from build123d import *

# Parameters (mm, degrees)
BOSS_EXTRUDE1_DEPTH = 5
SKETCH2_R           = 1.5
CUT_EXTRUDE1_DEPTH  = 15.5
CUT_EXTRUDE3_DEPTH  = 27
CIRPATTERN1_COUNT   = 3
CIRPATTERN2_COUNT   = 3
SCALE_RATIO_1_SCALE = 1.3
SKETCH5_R           = 5
CUT_EXTRUDE4_DEPTH  = 10
CHAMFER1_SIZE       = 0.5
SKETCH8_R           = 2
CUT_EXTRUDE5_DEPTH  = 10
CHAMFER2_SIZE       = 0.5
FILLET1_R           = 0.5


with BuildPart() as part:
    # Sketch1 → Boss-Extrude1 (new body)
    with BuildSketch(Plane.XY):
        with BuildLine():
            Line((-26.5, -17.60918321), (-12.640472866, -9.607381488))
            ThreePointArc((-12.640472866, -9.607381488), (-13.75, -7.938566201), (-14.640472866, -6.143279873))
            Line((-14.640472866, -6.143279873), (-28.5, -14.145081595))
            Line((-28.5, -14.145081595), (-29.75, -11.980018086))
            Line((-29.75, -11.980018086), (-15.436166994, -3.715922747))
            ThreePointArc((-15.436166994, -3.715922747), (-13.75, 7.938566201), (-4.5, 15.226074127))
            Line((-4.5, 15.226074127), (-4.5, 31.754264805))
            Line((-4.5, 31.754264805), (-2, 31.754264805))
            Line((-2, 31.754264805), (-2, 15.750661362))
            ThreePointArc((-2, 15.750661362), (0, 15.877132403), (2, 15.750661362))
            Line((2, 15.750661362), (2, 31.754264805))
            Line((2, 31.754264805), (4.5, 31.754264805))
            Line((4.5, 31.754264805), (4.5, 15.226074127))
            ThreePointArc((4.5, 15.226074127), (13.75, 7.938566201), (15.436166994, -3.715922747))
            Line((15.436166994, -3.715922747), (29.75, -11.980018086))
            Line((29.75, -11.980018086), (28.5, -14.145081595))
            Line((28.5, -14.145081595), (14.640472866, -6.143279873))
            ThreePointArc((14.640472866, -6.143279873), (13.75, -7.938566201), (12.640472866, -9.607381488))
            Line((12.640472866, -9.607381488), (26.5, -17.60918321))
            Line((26.5, -17.60918321), (25.25, -19.77424672))
            Line((25.25, -19.77424672), (10.936166994, -11.510151381))
            ThreePointArc((10.936166994, -11.510151381), (0, -15.877132403), (-10.936166994, -11.510151381))
            Line((-10.936166994, -11.510151381), (-25.25, -19.77424672))
            Line((-25.25, -19.77424672), (-26.5, -17.60918321))
        make_face()
    extrude(amount=BOSS_EXTRUDE1_DEPTH)

    # Sketch2 → Cut-Extrude1 (cut, symmetric)
    with BuildSketch(Plane(origin=(0, 0, 0), x_dir=(0, 0, -1), z_dir=(1, 0, 0))):
        with Locations(Location((-2.5, 21, 0), (0, 0, 90))):
            Circle(SKETCH2_R)
    cut_extrude1 = extrude(amount=CUT_EXTRUDE1_DEPTH, both=True, mode=Mode.SUBTRACT)

    # Sketch4 → Cut-Extrude3 (cut)
    with BuildSketch(Plane.ZY.offset(4.5)):
        with BuildLine():
            Line((0, 21), (0, 31.754264805))
            Line((0, 31.754264805), (5, 31.754264805))
            Line((5, 31.754264805), (5, 21))
            ThreePointArc((5, 21), (2.5, 23.5), (0, 21))
        make_face()
    cut_extrude3 = extrude(amount=-CUT_EXTRUDE3_DEPTH, mode=Mode.SUBTRACT)

    # CirPattern1: Cut-Extrude3 ×3 about axis
    cirpattern1_axis = Axis((0, 0, 5), (0, 0, -1))
    for i in range(1, CIRPATTERN1_COUNT):
        add(cut_extrude3.rotate(cirpattern1_axis, i * 360 / CIRPATTERN1_COUNT), mode=Mode.SUBTRACT)

    # CirPattern2: Cut-Extrude1 ×3 about axis
    cirpattern2_axis = Axis((0, 0, 5), (0, 0, -1))
    for i in range(1, CIRPATTERN2_COUNT):
        add(cut_extrude1.rotate(cirpattern2_axis, i * 360 / CIRPATTERN2_COUNT), mode=Mode.SUBTRACT)


with BuildPart() as part_1:
    # Scale ratio 1: scaled about (0, 0, 2.5)
    add(part.part.scale(SCALE_RATIO_1_SCALE).moved(Location((0, 0, -0.75))))

    # Sketch5 → Cut-Extrude4 (cut)
    with BuildSketch(Plane.XY.offset(5.75)):
        Circle(SKETCH5_R)
    extrude(amount=-CUT_EXTRUDE4_DEPTH, mode=Mode.SUBTRACT)

    # Chamfer1
    chamfer1_edges = [part_1.edges().sort_by_distance(p)[0] for p in [
        (-5, 0, -0.75),
        (-5, 0, 5.75),
    ]]
    chamfer(chamfer1_edges, length=CHAMFER1_SIZE)

    # Sketch8 → Cut-Extrude5 (cut)
    with BuildSketch(Plane.XY.offset(5.75)):
        with Locations((0, 15)):
            Circle(SKETCH8_R)
        with Locations((12.990381057, -7.5)):
            Circle(SKETCH8_R)
        with Locations((-12.990381057, -7.5)):
            Circle(SKETCH8_R)
    extrude(amount=-CUT_EXTRUDE5_DEPTH, mode=Mode.SUBTRACT)

    # Chamfer2
    chamfer2_edges = [part_1.edges().sort_by_distance(p)[0] for p in [
        (-2, 15, -0.75),
        (-2, 15, 5.75),
        (10.990381057, -7.5, -0.75),
        (10.990381057, -7.5, 5.75),
        (-14.990381057, -7.5, -0.75),
        (-14.990381057, -7.5, 5.75),
    ]]
    chamfer(chamfer2_edges, length=CHAMFER2_SIZE)

    # Fillet1
    fillet1_edges = [part_1.edges().sort_by_distance(p)[0] for p in [
        (-16.432614725, -12.489595935, 2.5),
        (-19.032614725, -7.986263835, 2.5),
        (-20.067017093, -4.830699571, 2.5),
        (-5.85, 19.793896366, 2.5),
        (-2.6, 20.47585977, 2.5),
        (2.6, 20.47585977, 2.5),
        (5.85, 19.793896366, 2.5),
        (20.067017093, -4.830699571, 2.5),
        (19.032614725, -7.986263835, 2.5),
        (16.432614725, -12.489595935, 2.5),
        (14.217017093, -14.963196795, 2.5),
        (-14.217017093, -14.963196795, 2.5),
    ]]
    fillet(fillet1_edges, radius=FILLET1_R)


solid = part_1.part
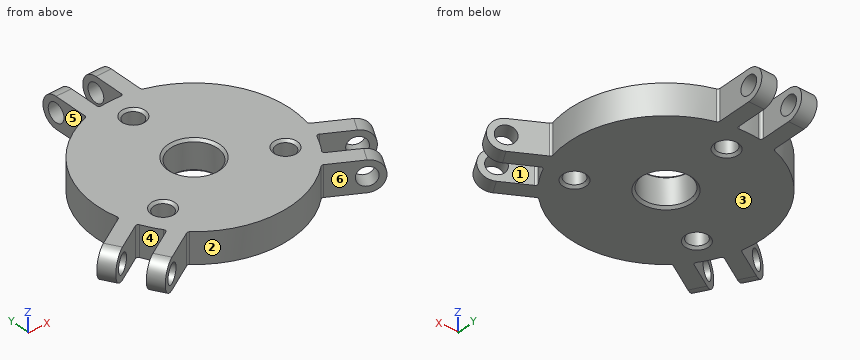
The listing builds one solid part. Answer for the finished solid, in the listing's coordinates (mm). Face numbers are marked on the shaded views. A direction names the side the tool comes from. Round coordinates to 2 decimals unless told otherwise and drop trailing zeros. Write each loop counter-clockwise with the first axis right and the second up, starting at its lowest first coordinate (ties: lowest second). Pieces come first, ordered by that corner, then holes. Notation, with made-up numbers: M -31,-7.5 L 7,-7.5 A21 ccw 7,29.5 Z; hole C 22,37 d2. An arc over 180 degrees is marked long. Write each question's results on one line, items separated by ' | '. Start each with the question number.
Item 1: A cutting plane is placed at A-A on x = 0. Write down the section's boundary in (y, z).
Item 2: A cutting plane is placed at C-C on y = 15. Write down the section's boundary in (x, z).
Item 3: A cutting plane is placed at B-B on y = 22.5. Write down the section's boundary in (x, z).
Item 4: For the marked faces 4, 5 and 6, determine the directions among +Z, -Z, +X, -X, +Y, -Y from which every point of the face is accessible in a straight line to the end or side of a thin tool.
Item 5: For a pull along Y with two mould halves and no side action, classify the marked faces 1, 2 and 3 as pulls with the +Y half, pulls with the -Y half, needs draft (parallel to the pull), parting line crosses it, or undercut.
Item 6: A cutting plane is placed at D-D on z = 3.5. State how many separate pieces and enclosed holes the cut face has, and give its area (3 significant figures).
Item 7: Straight lines are drawn through the part: L1, parallel to Y at x = 0, z = 2.8; L2, parallel to Y at x = 3, z = 3.5; L3, parallel to X at y = -11, z = 3.25. For each, find the intervals that lie inside material, in ascending order. Write a range as [from, to].
Item 8: Flat-ended cylindrical pins translate along their axes: pin 1 Ø3 at (y, z) = (27, 4) entering from -X; pin 2 Ø2.5 at (x, y) = (-12.99, -7.5) entering from -Z; pin 3 Ø2 at (y, z) = (-14, 5) entering from -X; pin 4 Ø11.5 at (x, y) = (0, 0) entering from -Z. Find the tip coordinate at first contact, or state that the pin passes through.
Check sheet entries:
1) outline: M -20.64,-0.75 L -5.5,-0.75 L -5,-0.25 L -5,5.25 L -5.5,5.75 L -20.64,5.75 Z; M 5,-0.25 L 5.5,-0.75 L 12.5,-0.75 L 13,-0.25 L 13,5.25 L 12.5,5.75 L 5.5,5.75 L 5,5.25 Z; M 17,-0.25 L 17.5,-0.75 L 20.64,-0.75 L 20.64,5.75 L 17.5,5.75 L 17,5.25 Z
2) outline: M -14.18,-0.75 L -2.5,-0.75 L -2,-0.25 L -2,5.25 L -2.5,5.75 L -14.18,5.75 Z; M 2,-0.25 L 2.5,-0.75 L 14.18,-0.75 L 14.18,5.75 L 2.5,5.75 L 2,5.25 Z
3) outline: M -5.85,-0.75 L -2.6,-0.75 L -2.6,5.75 L -5.85,5.75 Z; M 2.6,-0.75 L 5.85,-0.75 L 5.85,5.75 L 2.6,5.75 Z
4) face 4: +Z, -Z | face 5: +Z, -Z, -X, +Y | face 6: +Z, -Z, -Y
5) face 1: undercut | face 2: pulls with the -Y half | face 3: needs draft
6) separate pieces: 7 | enclosed holes: 4 | area: 1,360 mm²
7) L1: [-20.64, -5], [5, 13], [17, 20.64] | L2: [-20.42, -4], [4, 25.63], [28.97, 30.39] | L3: [-28.82, -27.25], [-17.46, 17.46], [27.25, 28.82]
8) pin 1: x = -5.85 | pin 2: through | pin 3: x = -20.78 | pin 4: z = -0.75
